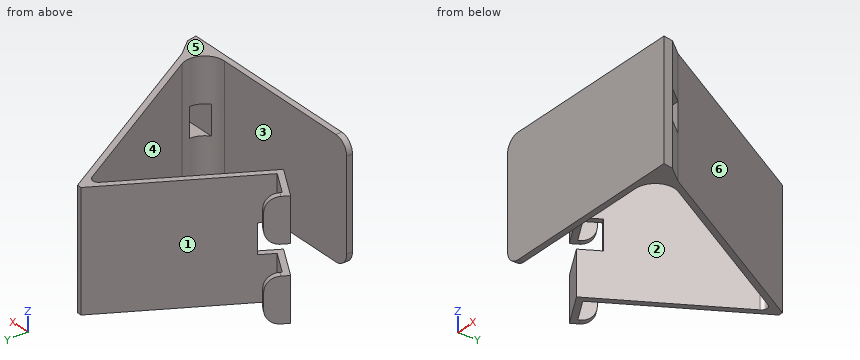
```python
from build123d import *

# Parameters (mm, degrees)
STAND_BODY_60MM_DEPTH = 30
CABLE_NOTCH_SKETCH_W  = 15
CABLE_NOTCH_SKETCH_H  = 8
CABLE_NOTCH_DEPTH     = 152.518975709
SLOT_15X11_REACH      = 167.253
SLOT_15X11_SKETCH_W   = 15
SLOT_15X11_SKETCH_H   = 11
SLOT_EDGE_FILLET_R7_R = 7
BEND_FILLET_R7_R      = 7


with BuildPart() as part:
    # Stand Profile Sketch → Stand Body 60mm (new, symmetric)
    with BuildSketch(Plane.XY):
        with BuildLine():
            Line((0, 0), (80.483339502, 0))
            ThreePointArc((80.483339502, 0), (89.143593539, 5), (89.143593539, 15))
            Line((89.143593539, 15), (40.934846062, 98.5))
            ThreePointArc((40.934846062, 98.5), (38.336769851, 100), (35.738693639, 98.5))
            Line((35.738693639, 98.5), (-1.719854476, 33.619891486))
            Line((-1.719854476, 33.619891486), (-19.906387956, 44.119891486))
            Line((-19.906387956, 44.119891486), (-14.406387956, 53.646170928))
            Line((-14.406387956, 53.646170928), (-11.808311744, 52.146170928))
            Line((-11.808311744, 52.146170928), (-15.808311744, 45.217967697))
            Line((-15.808311744, 45.217967697), (-2.817930688, 37.717967697))
            Line((-2.817930688, 37.717967697), (37.182069312, 107))
            Line((37.182069312, 107), (39.491470389, 107))
            Line((39.491470389, 107), (95.494446501, 10))
            Line((95.494446501, 10), (102.118365096, 2))
            Line((102.118365096, 2), (103, -3))
            Line((103, -3), (0, -3))
            Line((0, -3), (0, 0))
        make_face()
    extrude(amount=STAND_BODY_60MM_DEPTH, both=True)

    # Cable Notch Sketch → Cable Notch (cut, through all)
    with BuildSketch(Plane(origin=(0, 0, 0), x_dir=(0, 0, -1), z_dir=(1, 0, 0))):
        with Locations((0, 6)):
            Rectangle(CABLE_NOTCH_SKETCH_W, CABLE_NOTCH_SKETCH_H)
    extrude(amount=CABLE_NOTCH_DEPTH, mode=Mode.SUBTRACT)

    # Slot 15x11 Sketch → Slot 15x11 (cut, up to next)
    with BuildSketch(Plane(origin=(-34.034264386, 19.649691705, 0), x_dir=(0, 0, 1), z_dir=(-0.8660254037844446, 0.49999999999998995, 0)), mode=Mode.PRIVATE) as slot_15x11_sk1:
        with Locations((0, 33.755752861)):
            Rectangle(SLOT_15X11_SKETCH_W, SLOT_15X11_SKETCH_H)
    slot_15x11_tool1 = extrude(slot_15x11_sk1.sketch, amount=-SLOT_15X11_REACH, mode=Mode.PRIVATE) & part.part
    add(slot_15x11_tool1.solids().sort_by_distance((-17.156388, 48.883031, 0))[0], mode=Mode.SUBTRACT)

    # Slot Edge Fillet R7
    slot_edge_fillet_r7_edges = [part.edges().sort_by_distance(p)[0] for p in [
        (-13.10734985, 52.896170928, -30),
        (-13.10734985, 52.896170928, 30),
        (-13.10734985, 52.896170928, 7.5),
        (-13.10734985, 52.896170928, -7.5),
    ]]
    fillet(slot_edge_fillet_r7_edges, radius=SLOT_EDGE_FILLET_R7_R)

    # Bend Fillet R7
    bend_fillet_r7_edges = [part.edges().sort_by_distance(p)[0] for p in [
        (0, -1.5, -30),
        (0, -1.5, 30),
    ]]
    fillet(bend_fillet_r7_edges, radius=BEND_FILLET_R7_R)


solid = part.part
```
CAD build for the part. Positions are in the model's coordinates, mm. Face numbers are marked on the shaded views. A direction names the side the tool comes from. Round coordinates to 2 decimals unless told otherwise and drop trailing zeros. Order: outer loops, then holes, each group sorted by start corner. A loop starts at its lowest first (then second) coordinate and runs counter-clockwise, first axis right, second up. Notation, with made-up numbers: (-3, 38.5) - (43, 38.5) arc R30 cw to (43, 63.5) - close; hole circle Ø1 at (34, 50). An arc over 180 degrees is marked (long way). Answer in a Markdown table with one row per item. Add a question column.
(1) Probe L1, parallel to X at y = 47.5, z = -19; L2, parallel to Y at x = 66, z = 6.5; L3, parallel to X at y = 47, z = -16.5. List the from-to ranges inside material, lowest first. Write a range as [from, to].
(2) Band-saw the part on C-C on z = -17. List the corners of the cut face in (x, y), and give its area (3 significant figures).
(3) Drop flat-ended pins along their axis: pin 1 Ø5 at (x, z) = (82.5, -5) entering from +Y; pin 2 Ø6 at (x, z) = (-1, 5.5) entering from +Y; pin 3 Ø16.5 at (x, z) = (95.5, 3.5) entering from +Y. Give the stop position or say it passes through.
(4) 3-axis set-ups, long thin cutter, end or side, ignore diameter. For the marked faces 1, 2 and 3: which of +Z, -Z, +X, -X, +Y, -Y reach the whole face in a straight line?
(5) Band-saw the part on A-A on x = -10. List the corners of the cut face in (y, z), and give its area (3 significant figures).
(6) Mould opens along Y. For the marked faces 4, 5 and 6 say: +Y half, -Y half, draft (parallel to the pull), parting line (faces both ways), or undercut.
(7) Band-saw the part on B-B on y = 61. List the corners of the cut face in (x, z), and give its area (3 significant figures).
(8) Band-saw the part on D-D on y = 27. List the corners of the cut face in (x, z), and give its area (3 significant figures).
Data:
| question | item | result |
|---|---|---|
| 1 | L1 | x = [-17.95, -14.49], [2.83, 6.29], [70.38, 73.84] |
| 1 | L2 | y = [-3, 0], [55.09, 61.09] |
| 1 | L3 | x = [-18.24, -14.78], [2.54, 6.01], [70.67, 74.13] |
| 2 | outline | (-19.91, 44.12) - (-1.72, 33.62) - (35.74, 98.5) arc R3 cw to (40.93, 98.5) - (89.14, 15) arc R10 cw to (80.48, 0) - (0, 0) - (0, -3) - (103, -3) - (102.12, 2) - (95.49, 10) - (39.49, 107) - (37.18, 107) - (-2.82, 37.72) - (-15.81, 45.22) - (-11.81, 52.15) - (-14.41, 53.65) - close |
| 2 | area | 1,090 mm^2 |
| 3 | pin 1 | stops at y = 36.84 |
| 3 | pin 2 | stops at y = 46.06 |
| 3 | pin 3 | stops at y = 24.28 |
| 4 | face 1 | +Z, -Z, +Y |
| 4 | face 2 | +Z, -Z |
| 4 | face 3 | +Z, -Z, -X |
| 5 | outline | (38.4, -30) - (41.86, -30) - (41.86, -7.5) - (38.4, -7.5) - close; (38.4, 7.5) - (41.86, 7.5) - (41.86, 30) - (38.4, 30) - close |
| 5 | area | 156 mm^2 |
| 6 | face 4 | undercut |
| 6 | face 5 | draft |
| 6 | face 6 | +Y half |
| 7 | outline | (10.62, -30) - (14.09, -30) - (14.09, 30) - (10.62, 30) - close; (62.59, -30) - (66.05, -30) - (66.05, 30) - (62.59, 30) - close |
| 7 | area | 416 mm^2 |
| 8 | outline | (82.22, -30) - (85.68, -30) - (85.68, 30) - (82.22, 30) - close |
| 8 | area | 208 mm^2 |
